Build history of the part. All positions in model axes, mm. A direction names the side the tool comes from. Give positions to 0.01 mm unless a question says otherwise; leave off trailing zeros. Loops run counter-clockwise (first coordinate to the right, second up) from the corner with the lowest first, then second, coordinate; pieces in that order, holes last. Notation, with made-up numbers: (-34.75, -29) -> (-16.75, -29) arc R22 cw to (-16.75, 1) -> close; hole circle Ø1 at (18, -7). An arc over 180 degrees is marked (long way). Answer as a JSON object with one key per item and string values. Group by question number.
from build123d import *

# Parameters (mm, degrees)
WEB_PLATE_PROFILE_R          = 5
WEB_PLATE_PROFILE_R_2        = 2.5
WEB_PLATE_EXTRUDE_10MM_DEPTH = 5


with BuildPart() as part:
    # Web Plate Profile → Web Plate Extrude 10mm (new, symmetric)
    with BuildSketch(Plane(origin=(0, 0, 0), x_dir=(1, 0, 0), z_dir=(0, 1, 0))):
        with BuildLine():
            Line((-6, 4), (-6, 66.252272915))
            ThreePointArc((-6, 66.252272915), (-5.740251485, 93.858192988), (13.963751735, 74.52152964))
            Line((13.963751735, 74.52152964), (74.52152964, 13.963751735))
            ThreePointArc((74.52152964, 13.963751735), (93.858192988, -5.740251485), (66.252272915, -6))
            Line((66.252272915, -6), (4, -6))
            ThreePointArc((4, -6), (-3.071067812, -3.071067812), (-6, 4))
        make_face()
        with Locations(Location((0, 80, 0), (0, 0, 270))):
            Circle(WEB_PLATE_PROFILE_R, mode=Mode.SUBTRACT)
        with Locations(Location((80, 0, 0), (0, 0, 270))):
            Circle(WEB_PLATE_PROFILE_R, mode=Mode.SUBTRACT)
        with Locations(Location((4, 4, 0), (0, 0, 270))):
            Circle(WEB_PLATE_PROFILE_R_2, mode=Mode.SUBTRACT)
        with Locations(Location((50, 0, 0), (0, 0, 270))):
            Circle(WEB_PLATE_PROFILE_R_2, mode=Mode.SUBTRACT)
        with Locations(Location((24, 0, 0), (0, 0, 270))):
            Circle(WEB_PLATE_PROFILE_R_2, mode=Mode.SUBTRACT)
        with Locations(Location((0, 24, 0), (0, 0, 270))):
            Circle(WEB_PLATE_PROFILE_R_2, mode=Mode.SUBTRACT)
        with Locations(Location((0, 50, 0), (0, 0, 270))):
            Circle(WEB_PLATE_PROFILE_R_2, mode=Mode.SUBTRACT)
        with Locations(Location((28.284271247, 51.715728753, 0), (0, 0, 270))):
            Circle(WEB_PLATE_PROFILE_R_2, mode=Mode.SUBTRACT)
        with Locations(Location((51.715728753, 28.284271247, 0), (0, 0, 270))):
            Circle(WEB_PLATE_PROFILE_R_2, mode=Mode.SUBTRACT)
        with BuildLine():
            Line((11.121320344, 60.393398282), (60.393398282, 11.121320344))
            ThreePointArc((60.393398282, 11.121320344), (61.043716536, 7.851949703), (58.272077939, 6))
            Line((58.272077939, 6), (15.588457268, 6))
            ThreePointArc((15.588457268, 6), (14.088457268, 6.401923789), (12.990381057, 7.5))
            ThreePointArc((12.990381057, 7.5), (10.606601718, 10.606601718), (7.5, 12.990381057))
            ThreePointArc((7.5, 12.990381057), (6.401923789, 14.088457268), (6, 15.588457268))
            Line((6, 15.588457268), (6, 58.272077939))
            ThreePointArc((6, 58.272077939), (7.851949703, 61.043716536), (11.121320344, 60.393398282))
        make_face(mode=Mode.SUBTRACT)
    extrude(amount=WEB_PLATE_EXTRUDE_10MM_DEPTH, both=True)


solid = part.part
(1) Pull direction X, two halves, no side cores. Call faces 1 (the cylindrical face through (-2.99, 0.07, 3.15)), 2 (the flat face through (32, 5, -40)), 3 (the cylindrical face through (49.275, -0.07, -28.826)), 4 (the cylindrical face through (47.56, -0.07, -0.54)): pulls with the +X half, pulls with the -X half, needs draft (parallel to the pull), parting line crosses it, or undercut.
(2) Saw through at D-D on x = 0. List the corners of the cut face in (y, z), plus the area to 3 significant figures.
(3) Pin check, flat tips, straight feed: pin 1 (3 mm diameter, centred on x = 38.5, y = -2.5, fed in from +Z); pin 2 (4 mm diameter, centred on x = 68, y = -2, fed in from -Z); pin 3 (5 mm diameter, centred on y = 2.5, z = -27, fed in from +X). Stop position of each tip, or through.
(4) Probe line 1 along X through (y, z) = (3, 1); line 2 along X through (y, z) = (-2.25, 0); line 3 along X through (y, z) = (4.5, -80). List the from-to ranges inside material, lowest first. Write a range as [from, to].
(5) 3-axis set-ups, long thin cutter, end or side, ignore diameter. For faces 5 (the flat face through (-6, 0, -35)), 6 (the flat face through (6, 0, -37)): which of +Z, -Z, +X, -X, +Y, -Y reach the whole face in a straight line?
(6) Saw through at B-B on x = 19.5. List the corners of the cut face in (y, z), plus the area to 3 significant figures.
(7) Saw through at C-C on z = -24. List the corners of the cut face in (x, y), plus the area to 3 significant figures.
(8) Saw through at A-A on z = 0. List the corners of the cut face in (x, y).
Calculated:
{
 "1": {"face 1": "pulls with the -X half", "face 2": "needs draft", "face 3": "undercut", "face 4": "undercut"},
 "2": {"outline": "(-5, -95) -> (5, -95) -> (5, -85) -> (-5, -85) -> close; (-5, -75) -> (5, -75) -> (5, -52.5) -> (-5, -52.5) -> close; (-5, -47.5) -> (5, -47.5) -> (5, -26.5) -> (-5, -26.5) -> close; (-5, -21.5) -> (5, -21.5) -> (5, 5.17) -> (-5, 5.17) -> close", "area": "802 mm^2"},
 "3": {"pin 1": "stops at z = 6", "pin 2": "stops at z = -22.49", "pin 3": "stops at x = 63.99"},
 "4": {"line 1": "x = [-4.66, 21.71], [26.29, 47.71], [52.29, 75.1], [84.9, 94.97]", "line 2": "x = [-5.17, 21.5], [26.5, 47.5], [52.5, 75], [85, 95]", "line 3": "x = [-15, -5], [5, 15]"},
 "5": {"face 5": "+Z, -X, +Y, -Y", "face 6": "+Y, -Y"},
 "6": {"outline": "(-5, -68.99) -> (5, -68.99) -> (5, -52.01) -> (-5, -52.01) -> close; (-5, -6) -> (5, -6) -> (5, 6) -> (-5, 6) -> close", "area": "290 mm^2"},
 "7": {"outline": "(-6, -5) -> (-2.5, -5) -> (-2.5, 5) -> (-6, 5) -> close; (2.5, -5) -> (6, -5) -> (6, 5) -> (2.5, 5) -> close; (47.51, -5) -> (64.49, -5) -> (64.49, 5) -> (47.51, 5) -> close", "area": "240 mm^2"},
 "8": {"outline": "(-5.17, -5) -> (21.5, -5) -> (21.5, 5) -> (-5.17, 5) -> close; (26.5, -5) -> (47.5, -5) -> (47.5, 5) -> (26.5, 5) -> close; (52.5, -5) -> (75, -5) -> (75, 5) -> (52.5, 5) -> close; (85, -5) -> (95, -5) -> (95, 5) -> (85, 5) -> close"}
}
